CAD build for the part. Positions are in the model's coordinates, mm. A direction names the side the tool comes from. Coordinates: 2 decimals unless noted, no trailing zeros. Loops run counter-clockwise (first coordinate to the right, second up) from the corner with the lowest first, then second, coordinate; pieces in that order, holes last.
1) Pin check, flat tips, straight feed: pin 1 Ø8 at (x, y) = (17, 24) entering from +Z; pin 2 Ø1.5 at (x, z) = (23, -11.5) entering from +Y; pin 3 Ø6 at (x, z) = (9.5, 19.5) entering from +Y. Stop position of each tip, or through.
2) Saw through at D-D, the plane z = -32. Write the cut outline in (x, y).
3) Saw through at A-A, the plane y = 0. Write the cut outline in (x, z), and give its area (3 significant figures).
4) Which spindle directions (+Z, -Z, +X, -X, +Y, -Y) get a long thin tool onto all of the face, cutting with end or side? Do faces 5 (the cylindrical face through (3.042, 15.703, 37.874)), 6 (the cylindrical face through (17.154, -25.296, 16.128)). Say none if no direction does.
5) Wall check: line 1 along Y through (x, z) = (16.5, 0); line 2 along X through (y, z) = (-34, -1.5); line 3 along Y through (x, z) = (21, -20.5). Give the ranges that are in metal, low to high.
6) Saw through at C-C, the plane x = 10. Write the cut outline in (y, z), and give its area (3 significant figures).
7) Two-plate mould, pull along X, no slides. Class faces 1 (the flat face through (34, 18, -19)), 2 (the flat face through (6, 30.2, 2.8)), 3 (the cylindrical face through (31.042, 15.703, 37.874)), 4 (the flat face through (28, 30.2, -2.8)): +X half, -X half, draft (parallel to the pull), parting line (faces both ways), or undercut.
```python
from build123d import *


with BuildPart() as part:
    # 草图1 → 旋转1 (revolve)
    with BuildSketch(Plane.XY, mode=Mode.PRIVATE) as revolve_1_sk:
        Polygon((0, 25), (0, 41), (6, 41), (6, 30), (28, 30), (28, 41), (34, 41), (34, 25), align=None)
    revolve(revolve_1_sk.sketch.rotate(Axis((0, 0, 0), (1, 0, 0)), 90), axis=Axis((0, 0, 0), (1, 0, 0)))


solid = part.part
```
Data:
1. pin 1: stops at z = 22.36
1. pin 2: stops at y = 28.01
1. pin 3: stops at y = 25.05
2. outline: (0, -25.63) - (6, -25.63) - (6, 25.63) - (0, 25.63) - close; (28, -25.63) - (34, -25.63) - (34, 25.63) - (28, 25.63) - close
3. outline: (0, -41) - (6, -41) - (6, -30) - (28, -30) - (28, -41) - (34, -41) - (34, -25) - (0, -25) - close; (0, 25) - (34, 25) - (34, 41) - (28, 41) - (28, 30) - (6, 30) - (6, 41) - (0, 41) - close
3. area: 604 mm2
4. face 5: +X, -X
4. face 6: none
5. line 1: y = -30 to -25, 25 to 30
5. line 2: x = 0 to 6, 28 to 34
5. line 3: y = -21.9 to -14.31, 14.31 to 21.9
6. outline: circle Ø60 at (0, 0); hole circle Ø50 at (0, 0)
6. area: 864 mm2
7. face 1: +X half
7. face 2: undercut
7. face 3: draft
7. face 4: undercut
